Build history of the part. All positions in model axes, mm. A direction names the side the tool comes from. Round coordinates to 2 decimals unless told otherwise and drop trailing zeros. Loops run counter-clockwise (first coordinate to the right, second up) from the corner with the lowest first, then second, coordinate; pieces in that order, holes last. Notation, with made-up numbers: (65, 26.5) - (92, 26.5) arc R22 cw to (92, 40.5) - close; hole circle Ø11 at (52.25, -23). An arc over 180 degrees is marked (long way). Put each result on its own line as item: value. Start each with the question number.
from build123d import *

# Parameters (mm, degrees)
SKETCH_1_W          = 80
SKETCH_1_H          = 42
EXTRUDE_1_DEPTH     = 10
SKETCH_2_W          = 46
SKETCH_2_H          = 42
CUT_EXTRUDE_1_DEPTH = 1.5
CHAMFER_1_SIZE      = 3
CUT_EXTRUDE_2_REACH = 47.97


with BuildPart() as part:
    # 草图1 → 凸台-拉伸1 (new body)
    with BuildSketch(Plane.XY):
        Rectangle(SKETCH_1_W, SKETCH_1_H)
    extrude(amount=EXTRUDE_1_DEPTH)

    # 草图2 → 切除-拉伸1 (cut)
    with BuildSketch(Plane.XY.offset(10)):
        Rectangle(SKETCH_2_W, SKETCH_2_H)
    extrude(amount=-CUT_EXTRUDE_1_DEPTH, mode=Mode.SUBTRACT)

    # 倒角1
    chamfer_1_edges = [part.edges().sort_by_distance(p)[0] for p in [
        (-40, 21, 5),
        (40, 21, 5),
    ]]
    chamfer(chamfer_1_edges, length=CHAMFER_1_SIZE)

    # 草图3 → 切除-拉伸2 (cut, up to next)
    with BuildSketch(Plane.XY.offset(8.5), mode=Mode.PRIVATE) as cut_extrude_2_sk1:
        with BuildLine():
            Line((-18.25, -14), (-18.25, -4))
            ThreePointArc((-18.25, -4), (-16, -1.75), (-13.75, -4))
            Line((-13.75, -4), (-13.75, -14))
            ThreePointArc((-13.75, -14), (-16, -16.25), (-18.25, -14))
        make_face()
    cut_extrude_2_tool1 = extrude(cut_extrude_2_sk1.sketch, amount=-CUT_EXTRUDE_2_REACH, mode=Mode.PRIVATE) & part.part
    cut_extrude_2 = cut_extrude_2_tool1.solids().sort_by_distance((-16, -9, 8.5))[0]
    add(cut_extrude_2, mode=Mode.SUBTRACT)

    # 镜向1: 切除-拉伸2 across plane
    add(cut_extrude_2.mirror(Plane(origin=(0, 0, 0), x_dir=(0, 0, 1), z_dir=(1, 0, 0))), mode=Mode.SUBTRACT)


solid = part.part
1) Slice it at D-D, the plane y = 4.5. Write the cut outline in (x, z), and give its area (3 significant figures).
2) Slice it at A-A, the plane y = -11. Write the cut outline in (x, z).
3) Slice it at C-C, the plane z = 0.75. Write the cut outline in (x, y).
4) Drop a flat-ended pin along its axis: pin 1 Ø6 at (x, y) = (16.5, 14) entering from +Z. Give the stop position or say it passes through.
5) Which spindle directions (+Z, -Z, +X, -X, +Y, -Y) get a long thin tool onto all of the face, cutting with end or side? Do faces 4 (the face through (31, 0, 10)), 5 (the face through (-23, 0, 9)), 6 (the face through (-18.25, -9, 4)). Say none if no direction does.
6) Pull direction X, two halves, no side cores. Call faces 1 (the face through (0, 0, 8.5)), 2 (the face through (40, -2, 5)), 3 (the face through (-32, 0, 10)): pulls with the +X half, pulls with the -X half, needs draft (parallel to the pull), parting line crosses it, or undercut.
7) Slice it at B-B, the plane x = -16. Write the cut outline in (y, z).
8) Drill centre lines: line 1 (X direction, y = -5, z = 3.5); line 2 (X direction, y = -16, z = 9.75); line 3 (Z direction, x = -14, y = 3). Where is each one in solid material? Low to high. Write a range as [from, to].
Taken from the geometry:
1. outline: (-40, 0) - (40, 0) - (40, 10) - (23, 10) - (23, 8.5) - (-23, 8.5) - (-23, 10) - (-40, 10) - close
1. area: 731 mm2
2. outline: (-40, 0) - (-18.25, 0) - (-18.25, 8.5) - (-23, 8.5) - (-23, 10) - (-40, 10) - close; (-13.75, 0) - (13.75, 0) - (13.75, 8.5) - (-13.75, 8.5) - close; (18.25, 0) - (40, 0) - (40, 10) - (23, 10) - (23, 8.5) - (18.25, 8.5) - close
3. outline: (-40, -21) - (40, -21) - (40, 18) - (37, 21) - (-37, 21) - (-40, 18) - close; hole (-18.25, -14) arc R2.25 ccw to (-13.75, -14) - (-13.75, -4) arc R2.25 ccw to (-18.25, -4) - close; hole (13.75, -14) arc R2.25 ccw to (18.25, -14) - (18.25, -4) arc R2.25 ccw to (13.75, -4) - close
4. pin 1: stops at z = 8.5
5. face 4: +Z, +X, -X, +Y, -Y
5. face 5: +Z, +Y, -Y
5. face 6: +Z, -Z
6. face 1: undercut
6. face 2: pulls with the +X half
6. face 3: needs draft
7. outline: (-21, 0) - (-16.25, 0) - (-16.25, 8.5) - (-21, 8.5) - close; (-1.75, 0) - (21, 0) - (21, 8.5) - (-1.75, 8.5) - close
8. line 1: x = [-40, -18.25], [-13.75, 13.75], [18.25, 40]
8. line 2: x = [-40, -23], [23, 40]
8. line 3: z = [0, 8.5]
